from build123d import *

# Parameters (mm, degrees)
BASE_RAIL_DEPTH                         = 170
BASE_RAIL_DEPTH_BACK                    = 100
UPRIGHT_BLOCK_PROFILE_SKETCH_R          = 15
UPRIGHT_BLOCK_WITH_SLOT_AND_HOLES_DEPTH = 120
UPRIGHT_EXTENSION_SKETCH_W              = 120
UPRIGHT_EXTENSION_SKETCH_H              = 10
UPRIGHT_EXTENSION_BLOCK_DEPTH           = 20
MOUNTING_SLOT_COUNTERBORE_10MM_DEPTH    = 10
MOUNTING_SLOT_THROUGH_REACH             = 208.155


with BuildPart() as part:
    # Base Rail Profile Sketch → Base Rail (new, two sides: drawn at the far end of the back side and taken through both)
    with BuildSketch(Plane.XY.offset(-BASE_RAIL_DEPTH_BACK)):
        Polygon((-46.010770255, 0), (46.010770255, 0), (60, 30), (60, 40), (-60, 40), (-60, 30), align=None)
    extrude(amount=BASE_RAIL_DEPTH + BASE_RAIL_DEPTH_BACK)

    # Upright Block Profile Sketch → Upright Block with Slot and Holes (add)
    with BuildSketch(Plane.XY):
        Polygon((-60, 40), (-60, 65), (-40, 140), (40, 140), (60, 65), (60, 40), align=None)
        with Locations((-26, 65)):
            Circle(UPRIGHT_BLOCK_PROFILE_SKETCH_R, mode=Mode.SUBTRACT)
        with Locations((26, 65)):
            Circle(UPRIGHT_BLOCK_PROFILE_SKETCH_R, mode=Mode.SUBTRACT)
        with BuildLine():
            Line((-24, 125), (24, 125))
            ThreePointArc((24, 125), (39, 110), (24, 95))
            Line((24, 95), (-24, 95))
            ThreePointArc((-24, 95), (-39, 110), (-24, 125))
        make_face(mode=Mode.SUBTRACT)
    extrude(amount=-UPRIGHT_BLOCK_WITH_SLOT_AND_HOLES_DEPTH)

    # Upright Extension Sketch → Upright Extension Block (add)
    with BuildSketch(Plane(origin=(0, 0, -100), x_dir=(-1, 0, 0), z_dir=(0, 0, -1))):
        with Locations((0, 35)):
            Rectangle(UPRIGHT_EXTENSION_SKETCH_W, UPRIGHT_EXTENSION_SKETCH_H)
    extrude(amount=UPRIGHT_EXTENSION_BLOCK_DEPTH)

    # Base Mounting Slot Sketch → Mounting Slot Counterbore 10mm (cut)
    with BuildSketch(Plane(origin=(0, 40, 0), x_dir=(1, 0, 0), z_dir=(0, 1, 0))):
        with BuildLine():
            Line((35, -50), (35, -105))
            ThreePointArc((35, -105), (0, -140), (-35, -105))
            Line((-35, -105), (-35, -50))
            ThreePointArc((-35, -50), (0, -15), (35, -50))
        make_face()
    extrude(amount=-MOUNTING_SLOT_COUNTERBORE_10MM_DEPTH, mode=Mode.SUBTRACT)

    # Sketch4_3 → Mounting Slot Through (cut, up to next)
    with BuildSketch(Plane(origin=(0, 40, 0), x_dir=(1, 0, 0), z_dir=(0, 1, 0)), mode=Mode.PRIVATE) as mounting_slot_through_sk1:
        with BuildLine():
            Line((16, -50), (16, -105))
            ThreePointArc((16, -105), (0, -121), (-16, -105))
            Line((-16, -105), (-16, -50))
            ThreePointArc((-16, -50), (0, -34), (16, -50))
        make_face()
    mounting_slot_through_tool1 = extrude(mounting_slot_through_sk1.sketch, amount=-MOUNTING_SLOT_THROUGH_REACH, mode=Mode.PRIVATE) & part.part
    add(mounting_slot_through_tool1.solids().sort_by_distance((0, 40, 77.5))[0], mode=Mode.SUBTRACT)


solid = part.part
Build history of the part. All positions in model axes, mm. A direction names the side the tool comes from. Coordinates: 2 decimals unless noted, no trailing zeros. Write each loop counter-clockwise with the first axis right and the second up, starting at its lowest first coordinate (ties: lowest second). Pieces come first, ordered by that corner, then holes.
(1) Drill centre lines: line 1 (Y direction, x = -26, z = -62); line 2 (Y direction, x = 22.5, z = -46); line 3 (Z direction, x = 25.5, y = 95). Where is each one in solid material? Low to high.
(2) Cut at A-A on x = 0. List the corners of the cut face in (y, z).
(3) Mould opens along Z. For faces 1 (the cylindrical face through (0, 15, 121)), 2 (the flat face through (0, 95, -59)), 3 (the flat face through (-1, 20, 170)), 4 (the flat face through (16, 15, 77)) say: pulls with the +Z half, pulls with the -Z half, needs draft (parallel to the pull), parting line crosses it, or undercut.
(4) Cut at C-C on y = 72. List the corners of the cut face in (x, z).
(5) Cut at D-D on z = -61. List the corners of the cut face in (x, y).
(6) Pin check, flat tips, straight feed: pin 1 Ø12 at (x, y) = (-20, 89) entering from +Z; pin 2 Ø24 at (y, z) = (13.5, 76.5) entering from +X; pin 3 Ø9 at (y, z) = (21.5, 87) entering from -X. Stop position of each tip, or through.
(7) 3-axis set-ups, long thin cutter, end or side, ignore diameter. For faces 5 (the flat face through (41, 40, 84)), 6 (the flat face through (-16, 15, 78)), 7 (the flat face through (35, 35, 77)), 8 (the flat face through (1, 30, -110)): which of +Z, -Z, +X, -X, +Y, -Y reach the whole face in a straight line?
(8) Cut at B-B on z = 87. List the corners of the cut face in (x, y), and give its area (3 significant figures).
Working result:
1. line 1: y = 0 to 50, 80 to 95.13, 124.87 to 140
1. line 2: y = 0 to 50.41, 79.59 to 95, 125 to 140
1. line 3: z = -120 to 0
2. outline: (0, -100) - (30, -100) - (30, -120) - (95, -120) - (95, 0) - (40, 0) - (40, 15) - (30, 15) - (30, 34) - (0, 34) - close; (0, 121) - (30, 121) - (30, 140) - (40, 140) - (40, 170) - (0, 170) - close; (125, -120) - (140, -120) - (140, 0) - (125, 0) - close
3. face 1: undercut
3. face 2: needs draft
3. face 3: pulls with the +Z half
3. face 4: undercut
4. outline: (-58.13, -120) - (-39.27, -120) - (-39.27, 0) - (-58.13, 0) - close; (-12.73, -120) - (12.73, -120) - (12.73, 0) - (-12.73, 0) - close; (39.27, -120) - (58.13, -120) - (58.13, 0) - (39.27, 0) - close
5. outline: (-60, 30) - (-46.01, 0) - (46.01, 0) - (60, 30) - (60, 65) - (40, 140) - (-40, 140) - (-60, 65) - close; hole circle Ø30 at (-26, 65); hole (-24, 95) - (24, 95) arc R15 ccw to (24, 125) - (-24, 125) arc R15 ccw to start; hole circle Ø30 at (26, 65)
6. pin 1: stops at z = 0
6. pin 2: stops at x = 57.9
6. pin 3: stops at x = -58.13
7. face 5: +Z, +X, -X, +Y
7. face 6: +Y, -Y
7. face 7: +Y
7. face 8: -Z, +X, -X, -Y
8. outline: (-60, 30) - (-46.01, 0) - (-16, 0) - (-16, 30) - (-35, 30) - (-35, 40) - (-60, 40) - close; (16, 0) - (46.01, 0) - (60, 30) - (60, 40) - (35, 40) - (35, 30) - (16, 30) - close
8. area: 2,720 mm2
